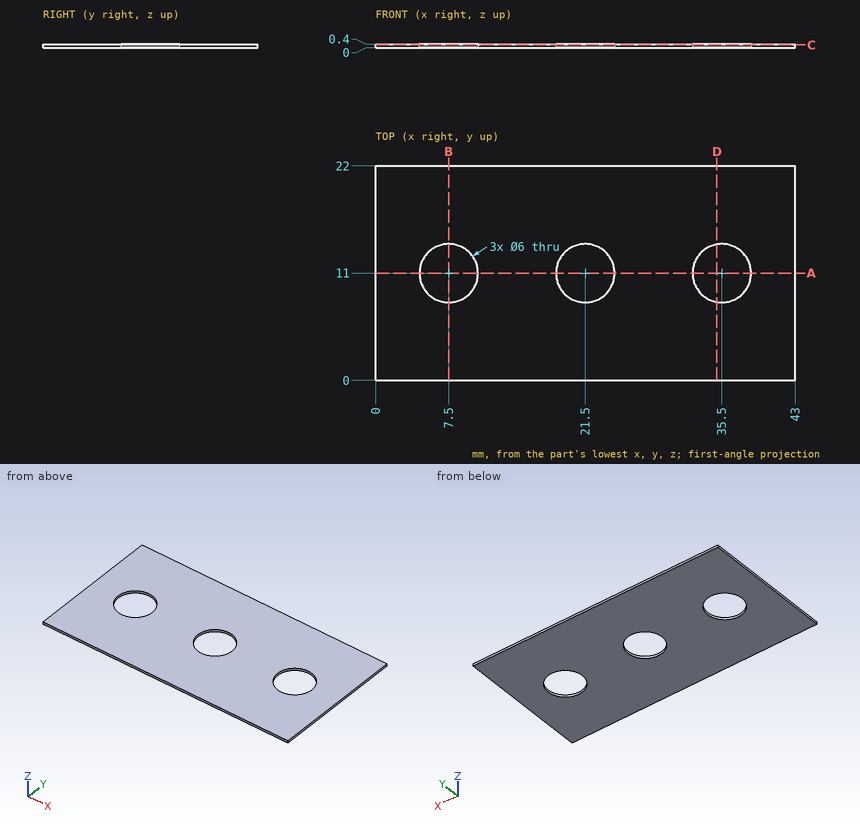
Geometry check sheet. Reference: drawing and pictorial views, mm from the part's lowest x, y, z. Give positions to 0.01 mm unless a question says otherwise; leave off trailing zeros. Loops run counter-clockwise (first coordinate to the right, second up) from the corner with the lowest first, then second, coordinate; pieces in that order, holes last. Notation, with made-up numbers: (11.5, 76.5) -> (25.5, 76.5) arc R17 ccw to (25.5, 93.5) -> close; hole circle Ø6 at (-11.75, 24.25). An arc over 180 degrees is marked (long way). Answer in a Markdown table with one row per item. Add a question column.
1) Cross-section at A-A on y = 11. Record the boundary of the cut face in (x, z).
2) Cross-section at D-D on x = 35. Record the boundary of the cut face in (y, z).
3) Material ranges on probe 1 along Y at (x, z) = (7.5, 0.2); probe 2 along X at (y, z) = (12.25, 0.15); probe 3 along Y at (x, z) = (10, 0.15), recorded low to high. Write a range as from..to.
4) Cross-section at C-C on z = 0.3. Record the boundary of the cut face in (x, y), and give its area (3 significant figures).
5) Gauge pin test, flat end, axial feed: P1, Ø9.5, axis at x = 21.5, y = 11, coming from the -Z side. Record the tip position at first contact, or that the pin passes through.
6) Cross-section at B-B on x = 7.5. Record the boundary of the cut face in (y, z), and give its area (3 significant figures).
Outcome:
| question | item | result |
|---|---|---|
| 1 | outline | (0, 0) -> (4.5, 0) -> (4.5, 0.4) -> (0, 0.4) -> close; (10.5, 0) -> (18.5, 0) -> (18.5, 0.4) -> (10.5, 0.4) -> close; (24.5, 0) -> (32.5, 0) -> (32.5, 0.4) -> (24.5, 0.4) -> close; (38.5, 0) -> (43, 0) -> (43, 0.4) -> (38.5, 0.4) -> close |
| 2 | outline | (0, 0) -> (8.04, 0) -> (8.04, 0.4) -> (0, 0.4) -> close; (13.96, 0) -> (22, 0) -> (22, 0.4) -> (13.96, 0.4) -> close |
| 3 | probe 1 | y = 0..8, 14..22 |
| 3 | probe 2 | x = 0..4.77, 10.23..18.77, 24.23..32.77, 38.23..43 |
| 3 | probe 3 | y = 0..9.34, 12.66..22 |
| 4 | outline | (0, 0) -> (43, 0) -> (43, 22) -> (0, 22) -> close; hole circle Ø6 at (7.5, 11); hole circle Ø6 at (21.5, 11); hole circle Ø6 at (35.5, 11) |
| 4 | area | 861 mm^2 |
| 5 | P1 | stops at z = 0 |
| 6 | outline | (0, 0) -> (8, 0) -> (8, 0.4) -> (0, 0.4) -> close; (14, 0) -> (22, 0) -> (22, 0.4) -> (14, 0.4) -> close |
| 6 | area | 6.40 mm^2 |
